from build123d import *

# Parameters (mm, degrees)
SKETCH1_W                   = 16
SKETCH1_H                   = 10
BOSS_EXTRUDE1_DEPTH         = 10
SKETCH2_W                   = 16
SKETCH2_H                   = 4
CUT_EXTRUDE1_DEPTH          = 10
SKETCH3_W                   = 10
SKETCH3_H                   = 10
BOSS_EXTRUDE2_DEPTH         = 7
SKETCH4_W                   = 2.5
SKETCH4_H                   = 10
BOSS_EXTRUDE3_DEPTH         = 4
SKETCH5_W                   = 6
SKETCH5_H                   = 4
CUT_EXTRUDE2_DEPTH          = 4
SKETCH6_R                   = 1
BOSS_EXTRUDE4_DEPTH         = 3
SKETCH7_R                   = 1.3
BOSS_EXTRUDE5_DEPTH         = 1
SKETCH8_W                   = 18
SKETCH8_H                   = 10
BOSS_EXTRUDE6_DEPTH         = 4
TAP_DRILL_FOR_M5_TAP1_D     = 4.2
TAP_DRILL_FOR_M5_TAP1_DEPTH = 60
TAP_DRILL_FOR_M5_TAP1_TIP   = 1.2618073


with BuildPart() as part:
    # Sketch1 → Boss-Extrude1 (new body)
    with BuildSketch(Plane(origin=(0, 0, 0), x_dir=(1, 0, 0), z_dir=(0, 1, 0))):
        Rectangle(SKETCH1_W, SKETCH1_H)
    extrude(amount=BOSS_EXTRUDE1_DEPTH)

    # Sketch2 → Cut-Extrude1 (cut)
    with BuildSketch(Plane(origin=(0, 0, -5), x_dir=(-1, 0, 0), z_dir=(0, 0, -1))):
        with Locations((-8, 5)):
            Rectangle(SKETCH2_W, SKETCH2_H)
    extrude(amount=-CUT_EXTRUDE1_DEPTH, mode=Mode.SUBTRACT)

    # Sketch3 → Boss-Extrude2 (add)
    with BuildSketch(Plane.ZY.offset(8)):
        with Locations((0, 5)):
            Rectangle(SKETCH3_W, SKETCH3_H)
    extrude(amount=BOSS_EXTRUDE2_DEPTH)

    # Sketch4 → Boss-Extrude3 (add)
    with BuildSketch(Plane(origin=(0, 0, -5), x_dir=(-1, 0, 0), z_dir=(0, 0, -1))):
        with Locations((13.75, 5)):
            Rectangle(SKETCH4_W, SKETCH4_H)
    boss_extrude3 = extrude(amount=BOSS_EXTRUDE3_DEPTH)

    # Mirror1: Boss-Extrude3 across plane
    add(boss_extrude3.mirror(Plane(origin=(0, 0, 0), x_dir=(1, 0, 0), z_dir=(0, 0, -1))))

    # Sketch5 → Cut-Extrude2 (cut)
    with BuildSketch(Plane(origin=(0, 0, 0), x_dir=(0, 0, -1), z_dir=(1, 0, 0))):
        with Locations((0, 5)):
            Rectangle(SKETCH5_W, SKETCH5_H)
    extrude(amount=-CUT_EXTRUDE2_DEPTH, mode=Mode.SUBTRACT)

    # Sketch6 → Boss-Extrude4 (add)
    with BuildSketch(Plane(origin=(-4, 0, 0), x_dir=(0, 0, -1), z_dir=(1, 0, 0))):
        with Locations((0, 5)):
            Circle(SKETCH6_R)
    extrude(amount=BOSS_EXTRUDE4_DEPTH)

    # Sketch7 → Boss-Extrude5 (add)
    with BuildSketch(Plane(origin=(-1, 0, 0), x_dir=(0, 0, -1), z_dir=(1, 0, 0))):
        with Locations((0, 5)):
            Circle(SKETCH7_R)
    extrude(amount=-BOSS_EXTRUDE5_DEPTH)

    # Sketch8 → Boss-Extrude6 (add)
    with BuildSketch(Plane.ZY.offset(15)):
        with Locations((0, 5)):
            Rectangle(SKETCH8_W, SKETCH8_H)
    extrude(amount=BOSS_EXTRUDE6_DEPTH)

    # Tap Drill for M5 Tap1
    with Locations(Plane.XZ):
        with Locations((-16, 0)):
            Hole(TAP_DRILL_FOR_M5_TAP1_D / 2, depth=TAP_DRILL_FOR_M5_TAP1_DEPTH)
            with Locations((0, 0, -(TAP_DRILL_FOR_M5_TAP1_DEPTH + TAP_DRILL_FOR_M5_TAP1_TIP / 2))):  # 118° drill point
                Cone(0, TAP_DRILL_FOR_M5_TAP1_D / 2, TAP_DRILL_FOR_M5_TAP1_TIP, mode=Mode.SUBTRACT)


solid = part.part
The listing builds one solid part. Answer for the finished solid, in the listing's coordinates (mm). A direction names the side the tool comes from. Coordinates: 2 decimals unless noted, no trailing zeros. Write each loop counter-clockwise with the first axis right and the second up, starting at its lowest first coordinate (ties: lowest second). Pieces come first, ordered by that corner, then holes. Notation, with made-up numbers: M 43,77.5 L 48,77.5 A24 cw 48,88.5 Z; hole C 29,87 d5. An arc over 180 degrees is marked long. Use one line per item in the form item = value.
Item 1: The mould has two halves that part along Z. Classify faces 4 (the face through (-2, 5, -5)), 5 (the face through (-12.5, 5, -7)), 6 (the face through (-2, 5, 3)): released by +Z, released by -Z, zero draft, split by the parting line, or undercut.
Model answer:
face_4 = released by -Z
face_5 = zero draft
face_6 = undercut
Item 2: Find section A-A, the plane x = 6. Give the vertices of the cut face in (y, z), plus the area to 3 significant figures.
Model answer:
outline = M 0,-5 L 3,-5 L 3,5 L 0,5 Z; M 7,-5 L 10,-5 L 10,5 L 7,5 Z
area = 60.0 mm2
Item 3: Find section B-B, the plane z = 0. Give the vertices of the cut face in (x, y), plus the area to 3 significant figures.
Model answer:
outline = M -19,0 L -18.1,0 L -18.1,10 L -19,10 Z; M -13.9,0 L 8,0 L 8,3 L -4,3 L -4,4 L -2,4 L -2,3.7 L -1,3.7 L -1,6.3 L -2,6.3 L -2,6 L -4,6 L -4,7 L 8,7 L 8,10 L -13.9,10 Z
area = 187 mm2
Item 4: For faces 1 (the face through (-12.5, 5, 7)), 2 (the face through (-1, 5, 0)), 3 (the face through (-3, 6, 0)), determine the directions among +Z, -Z, +X, -X, +Y, -Y from which every point of the face is accessible in a straight line to the end or side of a thin tool.
Model answer:
face_1 = +Z, +X, +Y, -Y
face_2 = +X
face_3 = none
Item 5: Find section C-C, the plane y = 5. Give the vertices of the cut face in (x, z), plus the area to 3 significant figures.
Model answer:
outline = M -19,-9 L -12.5,-9 L -12.5,-5 L 0,-5 L 0,-3 L -4,-3 L -4,-1 L -2,-1 L -2,-1.3 L -1,-1.3 L -1,1.3 L -2,1.3 L -2,1 L -4,1 L -4,3 L 0,3 L 0,5 L -12.5,5 L -12.5,9 L -19,9 Z; hole C -16,0 d4.2
area = 211 mm2
Item 6: Find the intervals of material crossed by probe 1 along Z at (x, y) = (-16, 7.5); probe 2 along Y at (x, z) = (4.5, 3.75); probe 3 along X at (y, z) = (4.5, 1.25), in increasing order.
Model answer:
probe_1 = -9 to -2.1, 2.1 to 9
probe_2 = 0 to 3, 7 to 10
probe_3 = -19 to -17.69, -14.31 to -4
Item 7: Find section D-D, the plane x = -16. Give the vertices of the cut face in (y, z).
Model answer:
outline = M 0,-9 L 10,-9 L 10,-2.1 L 0,-2.1 Z; M 0,2.1 L 10,2.1 L 10,9 L 0,9 Z
Item 8: Given P1, Ø0.8, axis at y = 5.5, z = 0.5, coming from the +X side; P2, Ø1.2, axis at x = -2, y = 5, coming from the -Z side; P3, Ø3, axis at y = 5.5, z = -7, coming from the +X side; P4, Ø3.5, axis at x = -16, z = 0, coming from the +Y side, each flat-ended and moving along its own axis, determine where each tip first touches the part or whether it passes through.
Model answer:
P1 = -1
P2 = -5
P3 = -12.5
P4 = through
